from build123d import *

# Parameters (mm, degrees)
SKETCH1_R             = 6
BOSS_EXTRUDE1_DEPTH   = 75
M5_TAPPED_HOLE1_D     = 4.2
M5_TAPPED_HOLE1_DEPTH = 12.4
M5_TAPPED_HOLE1_TIP   = 1.2618073
M5_TAPPED_HOLE2_D     = 4.2
M5_TAPPED_HOLE2_DEPTH = 12.4
M5_TAPPED_HOLE2_TIP   = 1.2618073
CHAMFER1_SIZE         = 0.5
SKETCH6_R             = 2.5
CUT_EXTRUDE1_DEPTH    = 17


with BuildPart() as part:
    # Sketch1 → Boss-Extrude1 (new body)
    with BuildSketch(Plane(origin=(0, 0, 0), x_dir=(0, 0, -1), z_dir=(1, 0, 0))):
        Circle(SKETCH1_R)
    extrude(amount=BOSS_EXTRUDE1_DEPTH)

    # M5 Tapped Hole1
    with Locations(Plane(origin=(75, 0, 0), x_dir=(0, 0, -1), z_dir=(1, 0, 0))):
        with Locations((0, 0)):
            Hole(M5_TAPPED_HOLE1_D / 2, depth=M5_TAPPED_HOLE1_DEPTH)
            with Locations((0, 0, -(M5_TAPPED_HOLE1_DEPTH + M5_TAPPED_HOLE1_TIP / 2))):  # 118° drill point
                Cone(0, M5_TAPPED_HOLE1_D / 2, M5_TAPPED_HOLE1_TIP, mode=Mode.SUBTRACT)

    # M5 Tapped Hole2
    with Locations(Plane.ZY):
        with Locations((0, 0)):
            Hole(M5_TAPPED_HOLE2_D / 2, depth=M5_TAPPED_HOLE2_DEPTH)
            with Locations((0, 0, -(M5_TAPPED_HOLE2_DEPTH + M5_TAPPED_HOLE2_TIP / 2))):  # 118° drill point
                Cone(0, M5_TAPPED_HOLE2_D / 2, M5_TAPPED_HOLE2_TIP, mode=Mode.SUBTRACT)

    # Chamfer1
    chamfer1_edges = [part.edges().sort_by_distance(p)[0] for p in [
        (0, 0, 6),
        (75, 0, 6),
    ]]
    chamfer(chamfer1_edges, length=CHAMFER1_SIZE)

    # Sketch6 → Cut-Extrude1 (cut, symmetric)
    with BuildSketch(Plane(origin=(0, 0, 0), x_dir=(1, 0, 0), z_dir=(0, 1, 0))):
        with Locations(Location((37.5, 0, 0), (0, 0, 270))):
            Circle(SKETCH6_R)
    extrude(amount=CUT_EXTRUDE1_DEPTH, both=True, mode=Mode.SUBTRACT)


solid = part.part
Design review of the part built by this model. Coordinates are the model's own, in mm. A direction names the side the tool comes from. Round coordinates to 2 decimals unless told otherwise and drop trailing zeros. Write each loop counter-clockwise with the first axis right and the second up, starting at its lowest first coordinate (ties: lowest second). Pieces come first, ordered by that corner, then holes. Notation, with made-up numbers: (0, -39) - (18, -39) arc R20 ccw to (18, -23) - close; hole circle Ø3 at (-40, 16.25). An arc over 180 degrees is marked (long way). Return JSON: item names as keys, results as strings. Group by question number.
Item 1: Insertion check: P1, Ø3, axis at x = 59, y = 3, coming from the -Z side; P2, Ø4.5, axis at x = 37.5, z = 0, coming from the -Y side; P3, Ø3, axis at x = 33.5, z = -2, coming from the +Y side; P4, Ø5, axis at x = 60, y = 1, coming from the -Z side. Each pin has a flat end and moves straight along its axis. Give the tip position at first contact, or say it passes through.
Item 2: We need section B-B on x = 37.5. Write out the cut boundary in (y, z).
Item 3: We need section A-A on x = 18. Write out the cut boundary in (y, z).
Item 4: For probe 1 along X at (y, z) = (5.25, 0); probe 2 along Y at (x, z) = (5.5, 0); probe 3 along X at (y, z) = (-5.5, 1), list the stretches that pass through material, from the lowest coordinate up. Write a range as [from, to].
Item 5: Machinability: for faces 1 (the face through (68.713, 0.631, 2.003)), 2 (the face through (0, -2.4, 0.1)), 3 (the face through (6.287, 0.631, -2.003)), which of the approach directions +Z, -Z, +X, -X, +Y, -Y give a long, thin tool a straight path to every point of the face, cutting with its end or side? Answer none if there is none.
Item 6: The part is to be moulded in two halves that separate along Y. For faces 4 (the face through (61.56, -0.14, -0.34)), 5 (the face through (36.98, -2.3, -5.54)), 6 (the face through (35.06, 0.08, -0.54)), say which applies: pulls with the +Y half, pulls with the -Y half, needs draft (parallel to the pull), parting line crosses it, or undercut.
Model answer:
{
 "1": {"P1": "stops at z = -5.81", "P2": "passes through", "P3": "stops at y = 5.98", "P4": "stops at z = -6"},
 "2": {"outline": "(-5.45, -2.5) arc R6 ccw to (5.45, -2.5) - close; (-5.45, 2.5) - (5.45, 2.5) arc R6 ccw to start"},
 "3": {"outline": "circle Ø12 at (0, 0)"},
 "4": {"probe 1": "x = [0, 35], [40, 75]", "probe 2": "y = [-6, -2.1], [2.1, 6]", "probe 3": "x = [0.09, 35.21], [39.79, 74.91]"},
 "5": {"face 1": "+X", "face 2": "+Z, -Z, -X, +Y, -Y", "face 3": "-X"},
 "6": {"face 4": "undercut", "face 5": "parting line crosses it", "face 6": "needs draft"}
}
